from build123d import *

# Parameters (mm, degrees)
BASE_BLOCK_SKETCH_W         = 20
BASE_BLOCK_SKETCH_H         = 65
BASE_BLOCK_DEPTH            = 40
ANGLED_CUT_30DEG_DEPTH      = 56.283360969
ANGLED_CUT_30DEG_DEPTH_BACK = 56.283360969
SIDE_PAD_DEPTH              = 5
PAD_TRIM_CUT_DEPTH          = 60.634302209
PAD_TRIM_CUT_DEPTH_BACK     = 5
PIN_HOLE_SKETCH_R           = 3.5
PIN_HOLE_7_DEPTH            = 5
LEVER_ARM_SKETCH_R          = 3
LEVER_ARM_DEPTH             = 5


with BuildPart() as part:
    # Base Block Sketch → Base Block (new body)
    with BuildSketch(Plane.XY):
        Rectangle(BASE_BLOCK_SKETCH_W, BASE_BLOCK_SKETCH_H)
    extrude(amount=BASE_BLOCK_DEPTH)

    # Angled Cut Sketch → Angled Cut 30deg (cut, two sides: drawn at the far end of the back side and taken through both)
    with BuildSketch(Plane(origin=(10, 0, 0), x_dir=(0, 0, -1), z_dir=(1, 0, 0)).offset(-ANGLED_CUT_30DEG_DEPTH_BACK)):
        Polygon((-12.679491924, 32.5), (-30, 2.5), (-30, -18.5), (-40, -18.5), (-40, 32.5), align=None)
    extrude(amount=ANGLED_CUT_30DEG_DEPTH + ANGLED_CUT_30DEG_DEPTH_BACK, mode=Mode.SUBTRACT)

    # Side Pad Sketch → Side Pad (add)
    with BuildSketch(Plane(origin=(10, 0, 0), x_dir=(0, 0, -1), z_dir=(1, 0, 0))):
        with BuildLine():
            Line((-40, -32.5), (15, -32.5))
            ThreePointArc((15, -32.5), (22, -25.5), (15, -18.5))
            Line((15, -18.5), (-40, -18.5))
            Line((-40, -18.5), (-40, -32.5))
        make_face()
    side_pad = extrude(amount=SIDE_PAD_DEPTH)

    # Side Pad Mirror: Side Pad across plane
    add(side_pad.mirror(Plane(origin=(0, 0, 0), x_dir=(0, 0, 1), z_dir=(1, 0, 0))))

    # Pad Trim Sketch → Pad Trim Cut (cut, two sides: drawn at the far end of the back side and taken through both)
    with BuildSketch(Plane(origin=(15, 0, 0), x_dir=(0, 0, -1), z_dir=(1, 0, 0)).offset(-PAD_TRIM_CUT_DEPTH_BACK)):
        with BuildLine():
            Line((-40, -18.5), (-40, -32.5))
            Line((-40, -32.5), (15, -32.5))
            ThreePointArc((15, -32.5), (22, -25.5), (15, -18.5))
            Line((15, -18.5), (-40, -18.5))
        make_face()
    extrude(amount=PAD_TRIM_CUT_DEPTH + PAD_TRIM_CUT_DEPTH_BACK, mode=Mode.SUBTRACT)

    # Pin Hole Sketch → Pin Hole Ø7 (cut)
    with BuildSketch(Plane(origin=(-10, 0, 0), x_dir=(0, 0, -1), z_dir=(1, 0, 0))):
        with Locations(Location((15, -25.5, 0), (0, 0, 90))):
            Circle(PIN_HOLE_SKETCH_R)
    extrude(amount=-PIN_HOLE_7_DEPTH, mode=Mode.SUBTRACT)

    # Lever Arm Sketch → Lever Arm (add)
    with BuildSketch(Plane(origin=(10, 0, 0), x_dir=(0, 0, -1), z_dir=(1, 0, 0))):
        with BuildLine():
            Line((-12.679491924, 32.5), (-12.679491924, -3.20749005))
            Line((-12.679491924, -3.20749005), (35.278835908, 19.155845491))
            ThreePointArc((35.278835908, 19.155845491), (39.154580126, 27.015077298), (32.320508076, 32.5))
            Line((32.320508076, 32.5), (-12.679491924, 32.5))
        make_face()
        with Locations(Location((32.320508076, 25.5, 0), (0, 0, 90))):
            Circle(LEVER_ARM_SKETCH_R, mode=Mode.SUBTRACT)
    extrude(amount=LEVER_ARM_DEPTH)


solid = part.part
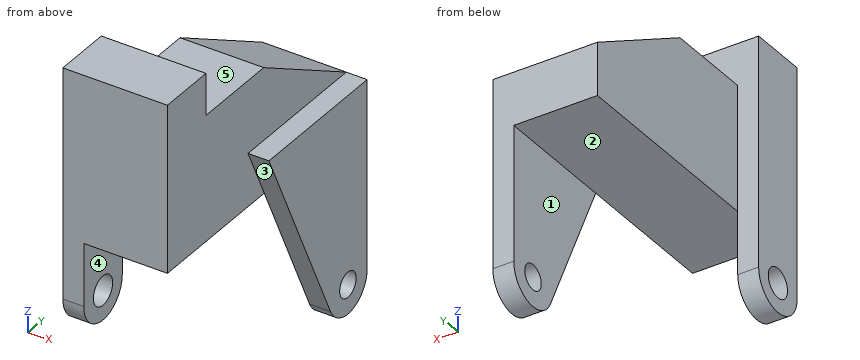
Geometry: final body of the model. Coordinates: model frame, mm. Face numbers are marked on the shaded views. A direction names the side the tool comes from. Give positions to 0.01 mm unless a question says otherwise; leave off trailing zeros. Write each loop counter-clockwise with the first axis right and the second up, starting at its lowest first coordinate (ties: lowest second). Pieces come first, ordered by that corner, then holes. Notation, with made-up numbers: M 84.25,60 L 127.25,60 A18 cw 127.25,95 Z; hole C 61.25,61.25 d5. An arc over 180 degrees is marked long. Answer in a Markdown table with one row per item. Add a question column.
(1) Reachability of the marked faces 1, 2, 3, 4 and 5 from +Z, -Z, +X, -X, +Y, -Y: full face, straight path, thin tool, end or side. Return the list, or none.
(2) Section D-D on z = -30.5. Return loops of the section in (x, y).
(3) Ray query, line 1 (Z direction, x = 13.95, y = 25.5); line 2 (Z direction, x = -13.9, y = -25.5); line 3 (X direction, y = -21, z = 29). Return the intervals inside material, ascending.
(4) Section C-C on x = 11.5. Return loops of the section in (y, z), and give its area (3 significant figures).
(5) Section B-B on y = -25.5. Return loops of the section in (x, z), and give its area (4 significant figures).
(6) Section A-A on z = -14. Return loops of the section in (x, y).
(7) First-contact query: pin 1 (2 mm diameter, centred on x = -10.5, z = 25, fed in from +Y); pin 2 (12 mm diameter, centred on y = -24.5, z = -11, fed in from +X); pin 3 (9 mm diameter, centred on y = 7.5, z = 9.5, fed in from -X); pin 4 (12 mm diameter, centred on y = 2, z = 14.5, fed in from +X). Flat tips, straight axial feed; report the tip coordinate or a pass-through.
Result set:
| question | item | result |
|---|---|---|
| 1 | face 1 | -Z, -X, +Y, -Y |
| 1 | face 2 | -Z, +Y, -Y |
| 1 | face 3 | -Z, +X, -Y |
| 1 | face 4 | -Z, +X, +Y, -Y |
| 1 | face 5 | +Z, +X, -X, +Y |
| 2 | outline | M 10,16.93 L 15,16.93 L 15,23.12 L 10,23.12 Z; M 10,27.88 L 15,27.88 L 15,32.5 L 10,32.5 Z |
| 3 | line 1 | z = -39.32 to -35.32, -29.32 to 12.68 |
| 3 | line 2 | z = -22 to -18.5, -11.5 to 40 |
| 3 | line 3 | x = -15 to 10 |
| 4 | outline | M -3.21,12.68 L 19.16,-35.28 A7 ccw 32.5,-32.32 L 32.5,12.68 Z; hole C 25.5,-32.32 d6 |
| 4 | area | 1,180 mm^2 |
| 5 | outline | M -15,-22 L -10,-22 L -10,-18.5 L -15,-18.5 Z; M -15,-11.5 L -10,-11.5 L -10,0 L 10,0 L 10,40 L -15,40 Z |
| 5 | area | 1,075 mm^2 |
| 6 | outline | M -15,-32.5 L -10,-32.5 L -10,-28.85 L -15,-28.85 Z; M -15,-22.15 L -10,-22.15 L -10,-18.5 L -15,-18.5 Z; M 10,9.23 L 15,9.23 L 15,32.5 L 10,32.5 Z |
| 7 | pin 1 | stops at y = 12.66 |
| 7 | pin 2 | stops at x = -10 |
| 7 | pin 3 | stops at x = -10 |
| 7 | pin 4 | stops at x = 15 |
